Geometry: final body of the model. Coordinates: model frame, mm. Face numbers are marked on the shaded views. A direction names the side the tool comes from. Round coordinates to 2 decimals unless told otherwise and drop trailing zeros. Loops run counter-clockwise (first coordinate to the right, second up) from the corner with the lowest first, then second, coordinate; pieces in that order, holes last. Notation, with made-up numbers: (-23, 72) - (-5, 72) arc R20 ccw to (-5, 107) - close; hole circle Ø7 at (75, -4). An arc over 180 degrees is marked (long way). Return JSON: item names as keys, results as strings. Group by question number.
1. Section B-B on z = -17.5. Return loops of the section in (x, y).
2. Material intervals for probe 1 along X at (y, z) = (3.5, -7); probe 2 along X at (y, z) = (42.5, -25); probe 3 along Y at (x, z) = (4.5, -12.5), sorted ascending.
3. Draft query along Z for the marked faces 1, 2 and 3. Return one class per face: +Z half, -Z half, draft (parallel to the pull), parting line (faces both ways), or undercut.
4. Section A-A on x = 11.75. Return loops of the section in (y, z), and give its area (3 significant figures).
5. First-contact query: pin 1 Ø12 at (x, z) = (17.5, -10.5) entering from -Y; pin 2 Ø12 at (x, y) = (22.5, 18.5) entering from -Z; pin 3 Ø4 at (y, z) = (26.5, -30) entering from +X; pin 4 Ø8 at (y, z) = (48.5, -20.5) entering from +X. Flat tips, straight axial feed; report the tip coordinate or a pass-through.
6. Section C-C on y = 65. Return loops of the section in (x, z), and give its area (3 significant figures).
7. Section D-D on x = 18. Return loops of the section in (y, z), and give its area (3 significant figures).
8. Set-up query: the marked faces 4, 5 and 6. Return all of +Z, -Z, +X, -X, +Y, -Y with unobstructed straight access to the full face (end or side cutting, diameter ignored); none if empty.
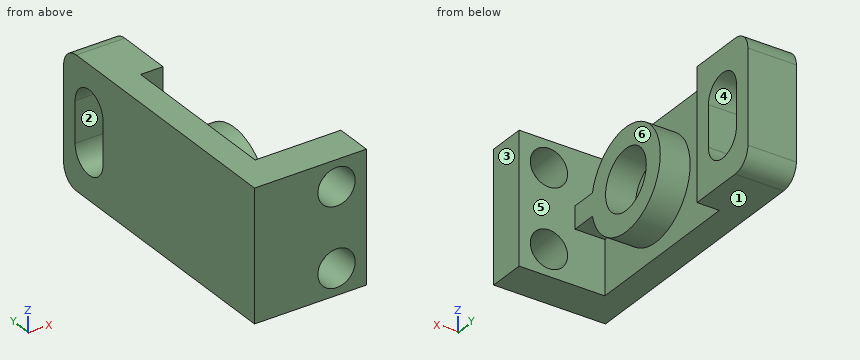
from build123d import *

# Parameters (mm, degrees)
BRACKET_BODY_DEPTH   = 35
BASE_HOLES_CUT_REACH = 81.687
BASE_HOLES_SKETCH_R  = 5
RING_BOSS_SKETCH_R   = 8
RING_BOSS_DEPTH      = 8
TOP_EDGE_FILLET_R5_R = 5
TOP_SLOT_CUT_REACH   = 86.493


with BuildPart() as part:
    # Bracket Profile Sketch → Bracket Body (new body)
    with BuildSketch(Plane.XY):
        Polygon((0, 0), (0, 75), (13, 75), (13, 55), (7, 55), (7, 10), (30, 10), (30, 0), align=None)
    extrude(amount=-BRACKET_BODY_DEPTH)

    # Base Holes Sketch → Base Holes Cut (cut, up to next)
    with BuildSketch(Plane(origin=(0, 10, 0), x_dir=(1, 0, 0), z_dir=(0, 1, 0)), mode=Mode.PRIVATE) as base_holes_cut_sk1:
        with Locations(Location((22, 28, 0), (0, 0, 270))):
            Circle(BASE_HOLES_SKETCH_R)
    base_holes_cut_tool1 = extrude(base_holes_cut_sk1.sketch, amount=-BASE_HOLES_CUT_REACH, mode=Mode.PRIVATE) & part.part
    # Base Holes Sketch → Base Holes Cut (cut, up to next)
    with BuildSketch(Plane(origin=(0, 10, 0), x_dir=(1, 0, 0), z_dir=(0, 1, 0)), mode=Mode.PRIVATE) as base_holes_cut_sk2:
        with Locations(Location((22, 7, 0), (0, 0, 270))):
            Circle(BASE_HOLES_SKETCH_R)
    base_holes_cut_tool2 = extrude(base_holes_cut_sk2.sketch, amount=-BASE_HOLES_CUT_REACH, mode=Mode.PRIVATE) & part.part
    add(base_holes_cut_tool1.solids().sort_by_distance((22, 10, -28))[0], mode=Mode.SUBTRACT)
    add(base_holes_cut_tool2.solids().sort_by_distance((22, 10, -7))[0], mode=Mode.SUBTRACT)

    # Ring Boss Sketch → Ring Boss (add)
    with BuildSketch(Plane(origin=(7, 0, 0), x_dir=(0, 0, -1), z_dir=(1, 0, 0))):
        with BuildLine():
            Line((14.5, 16.837553419), (14.5, 10))
            Line((14.5, 10), (20.5, 10))
            Line((20.5, 10), (20.5, 16.837553419))
            ThreePointArc((20.5, 16.837553419), (17.5, 43.5), (14.5, 16.837553419))
        make_face()
        with Locations(Location((17.5, 30, 0), (0, 0, 90))):
            Circle(RING_BOSS_SKETCH_R, mode=Mode.SUBTRACT)
    extrude(amount=RING_BOSS_DEPTH)

    # Top Edge Fillet R5
    top_edge_fillet_r5_edges = [part.edges().sort_by_distance(p)[0] for p in [
        (6.5, 75, -35),
        (6.5, 75, 0),
    ]]
    fillet(top_edge_fillet_r5_edges, radius=TOP_EDGE_FILLET_R5_R)

    # Top Slot Sketch → Top Slot Cut (cut, up to next)
    with BuildSketch(Plane(origin=(13, 0, 0), x_dir=(0, 0, -1), z_dir=(1, 0, 0)), mode=Mode.PRIVATE) as top_slot_cut_sk1:
        with BuildLine():
            Line((12, 70.5), (23, 70.5))
            ThreePointArc((23, 70.5), (28.5, 65), (23, 59.5))
            Line((23, 59.5), (12, 59.5))
            ThreePointArc((12, 59.5), (6.5, 65), (12, 70.5))
        make_face()
    top_slot_cut_tool1 = extrude(top_slot_cut_sk1.sketch, amount=-TOP_SLOT_CUT_REACH, mode=Mode.PRIVATE) & part.part
    add(top_slot_cut_tool1.solids().sort_by_distance((13, 65, -17.5))[0], mode=Mode.SUBTRACT)


solid = part.part
Taken from the geometry:
{
 "1": {"outline": "(0, 0) - (30, 0) - (30, 10) - (15, 10) - (15, 22) - (7, 22) - (7, 38) - (15, 38) - (15, 43.5) - (7, 43.5) - (7, 55) - (13, 55) - (13, 59.5) - (0, 59.5) - close; (0, 70.5) - (13, 70.5) - (13, 75) - (0, 75) - close"},
 "2": {"probe 1": "0 to 17, 27 to 30", "probe 2": "0 to 7", "probe 3": "0 to 59.5, 70.5 to 75"},
 "3": {"face 1": "-Z half", "face 2": "undercut", "face 3": "draft"},
 "4": {"outline": "(0, -35) - (10, -35) - (10, -20.5) - (16.84, -20.5) arc R13.5 ccw (long way) to (16.84, -14.5) - (10, -14.5) - (10, 0) - (0, 0) - close; (55, -35) - (70, -35) arc R5 ccw to (75, -30) - (75, -5) arc R5 ccw to (70, 0) - (55, 0) - close; hole circle Ø16 at (30, -17.5); hole (59.5, -23) arc R5.5 ccw to (70.5, -23) - (70.5, -12) arc R5.5 ccw to (59.5, -12) - close", "area": "1,230 mm2"},
 "5": {"pin 1": "y = 0", "pin 2": "through", "pin 3": "x = 15", "pin 4": "x = 7"},
 "6": {"outline": "(0, -35) - (13, -35) - (13, -28.5) - (0, -28.5) - close; (0, -6.5) - (13, -6.5) - (13, 0) - (0, 0) - close", "area": "169 mm2"},
 "7": {"outline": "(0, -35) - (10, -35) - (10, -31) - (0, -31) - close; (0, -25) - (10, -25) - (10, -10) - (0, -10) - close; (0, -4) - (10, -4) - (10, 0) - (0, 0) - close", "area": "230 mm2"},
 "8": {"face 4": "+X, -X", "face 5": "+X", "face 6": "+Z, -Z, +X, +Y"}
}
